Input: dimensioned drawing with shaded views. Units: mm. Origin: part minimum x, y, z. Coordinates: 2 decimals unless noted, no trailing zeros. Order: outer loops, then holes, each group sorted by start corner. A loop starts at its lowest first (then second) coordinate and runs counter-clockwise, first axis right, second up. Notation, with made-up numbers: (66, 1) -> (100, 1) arc R28 cw to (100, 34) -> close; hole circle Ø6 at (74.5, 53.25). An arc over 180 degrees is marked (long way). Write item = value, one per line. Start each with the question number.
Item 1: Mould query, pull axis X, two halves, no side actions, for the marked faces 1, 2 and 3. Classes: released by +X, released by -X, zero draft, split by the parting line, or undercut.
Item 2: Contact query for flat-ended pins moving along their axis: pin 1 (1.5 mm diameter, centred on x = 31, y = 7.5, fed in from +Z) (1 decimal); pin 2 (5 mm diameter, centred on x = 29, z = 15, fed in from -Y); pin 3 (8 mm diameter, centred on x = 17.5, y = 9, fed in from +Z). Output: stop coordinate, or through.
Item 3: Section query A-A (x = 6.5). Output: boundary loops of the cut face in (y, z) (1 decimal), then the cut area to 3 significant figures.
Item 4: Ray query, line 1 along X through (y, z) = (11, 16); line 2 along Z through (x, y) = (8.5, 15.25) (1 decimal); line 3 along Y through (x, z) = (31.5, 4.25) (1 decimal). Return the intervals inside material, ascending. Write a range as [from, to].
Item 5: Section query B-B (x = 24.5). Output: boundary loops of the cut face in (y, z), then the cut area to 3 significant figures.
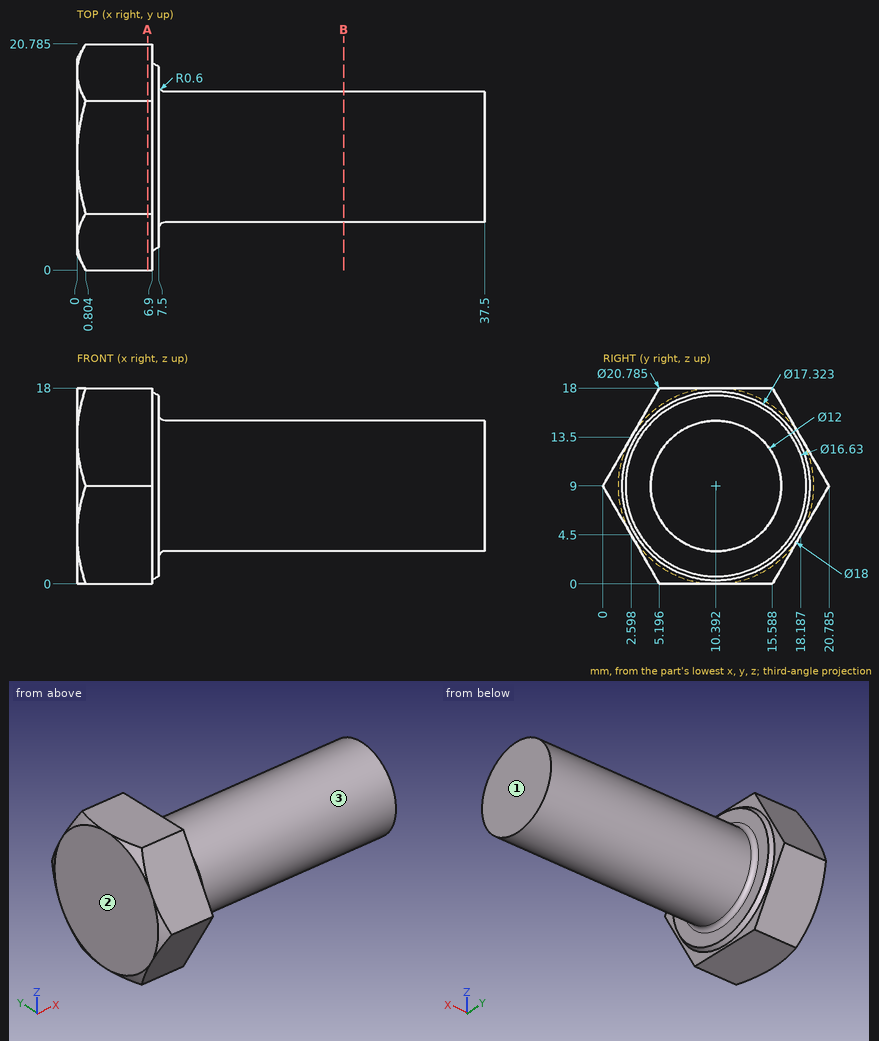
Computed:
q1.face_1 = released by +X
q1.face_2 = released by -X
q1.face_3 = zero draft
q2.pin_1 = 14.6
q2.pin_2 = 5.52
q2.pin_3 = 15
q3.outline = (0, 9) -> (5.2, 0) -> (15.6, 0) -> (20.8, 9) -> (15.6, 18) -> (5.2, 18) -> close
q3.area = 281 mm^2
q4.line_1 = [0, 7.5]
q4.line_2 = [5.5, 12.5]
q4.line_3 = [6.7, 14.1]
q5.outline = circle Ø12 at (10.39, 9)
q5.area = 113 mm^2
